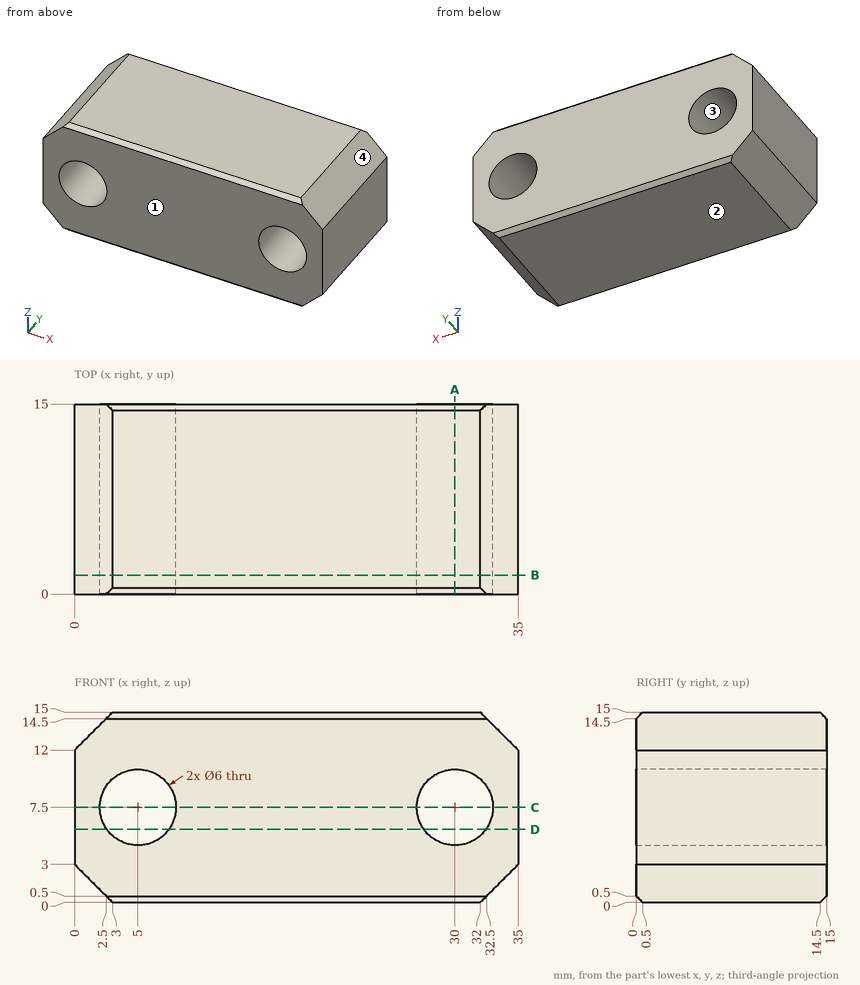
The drawing under review shows one solid part. Ordinate dimensions are in mm from its lowest x, y, z. Coordinates: 2 decimals unless noted, no trailing zeros. Order: outer loops, then holes, each group sorted by start corner. A loop starts at its lowest first (then second) coordinate and runs counter-clockwise, first axis right, second up. Notation, with made-up numbers: (-22.75, 8) -> (25.25, 8) arc R21 ccw to (25.25, 22) -> close; hole circle Ø11 at (11, -10). An arc over 180 degrees is marked (long way). Return JSON: item names as keys, results as strings.
1. We need section B-B on y = 1.5. Write out the cut boundary in (x, z), and give its area (3 significant figures).
Answer block:
{"outline": "(0, 3) -> (3, 0) -> (32, 0) -> (35, 3) -> (35, 12) -> (32, 15) -> (3, 15) -> (0, 12) -> close; hole circle Ø6 at (5, 7.5); hole circle Ø6 at (30, 7.5)", "area": "450 mm²"}
2. For line 1 (X direction, y = 11.5, z = 7.5); line 2 (X direction, y = 3.5, z = 5.25); line 3 (X direction, y = 1.5, z = 13.25), list the stretches that pass through material, from the lowest coordinate up. Write a range as from..to.
Answer block:
{"line 1": "0..2, 8..27, 33..35", "line 2": "0..3.02, 6.98..28.02, 31.98..35", "line 3": "1.25..33.75"}
3. We need section A-A on x = 30. Write out the cut boundary in (y, z).
Answer block:
{"outline": "(0, 0.5) -> (0.5, 0) -> (14.5, 0) -> (15, 0.5) -> (15, 4.5) -> (0, 4.5) -> close; (0, 10.5) -> (15, 10.5) -> (15, 14.5) -> (14.5, 15) -> (0.5, 15) -> (0, 14.5) -> close"}
4. We need section D-D on z = 5.75. Write out the cut boundary in (x, y), and give its area (3 significant figures).
Answer block:
{"outline": "(0, 0) -> (2.56, 0) -> (2.56, 15) -> (0, 15) -> close; (7.44, 0) -> (27.56, 0) -> (27.56, 15) -> (7.44, 15) -> close; (32.44, 0) -> (35, 0) -> (35, 15) -> (32.44, 15) -> close", "area": "379 mm²"}
5. We need section C-C on z = 7.5. Write out the cut boundary in (x, y).
Answer block:
{"outline": "(0, 0) -> (2, 0) -> (2, 15) -> (0, 15) -> close; (8, 0) -> (27, 0) -> (27, 15) -> (8, 15) -> close; (33, 0) -> (35, 0) -> (35, 15) -> (33, 15) -> close"}
6. The part is to be moulded in two halves that separate along Z. For the marked faces 1, 2, 3 and 4, say which applies: +Z half, -Z half, draft (parallel to the pull), parting line (faces both ways), or undercut.
Answer block:
{"face 1": "draft", "face 2": "-Z half", "face 3": "undercut", "face 4": "+Z half"}
